Model file for the job. Use its own axes, mm. Coordinates: 2 decimals unless noted, no trailing zeros. Order: outer loops, then holes, each group sorted by start corner. A loop starts at its lowest first (then second) coordinate and runs counter-clockwise, first axis right, second up.
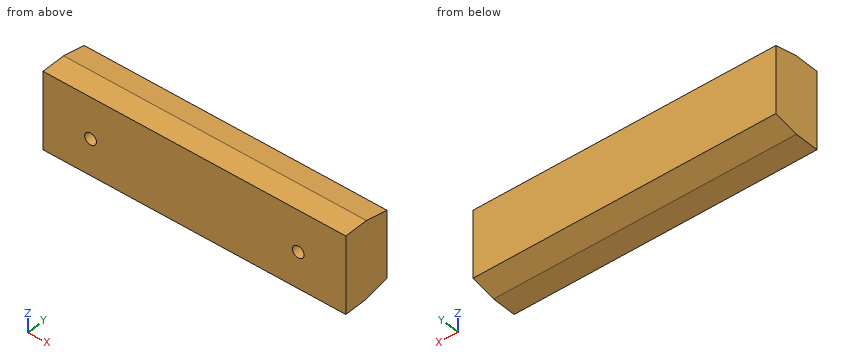
from build123d import *

# Parameters (mm, degrees)
SKETCH1_W             = 175
SKETCH1_H             = 28
BOSS_EXTRUDE1_DEPTH   = 45
M8_TAPPED_HOLE1_D     = 6.8
M8_TAPPED_HOLE1_DEPTH = 19.75
M8_TAPPED_HOLE1_TIP   = 2.042926105
CUT_EXTRUDE1_DEPTH    = 183.849665026


with BuildPart() as part:
    # Sketch1 → Boss-Extrude1 (new body)
    with BuildSketch(Plane.XY):
        with Locations((87.5, -14)):
            Rectangle(SKETCH1_W, SKETCH1_H)
    extrude(amount=BOSS_EXTRUDE1_DEPTH)

    # M8 Tapped Hole1
    with Locations(Plane(origin=(0, -28, 0), x_dir=(-1, 0, 0), z_dir=(0, -1, 0))):
        with Locations((-27.5, -21), (-147.5, -21)):
            Hole(M8_TAPPED_HOLE1_D / 2, depth=M8_TAPPED_HOLE1_DEPTH)
            with Locations((0, 0, -(M8_TAPPED_HOLE1_DEPTH + M8_TAPPED_HOLE1_TIP / 2))):  # 118° drill point
                Cone(0, M8_TAPPED_HOLE1_D / 2, M8_TAPPED_HOLE1_TIP, mode=Mode.SUBTRACT)

    # Sketch7 → Cut-Extrude1 (cut, through all)
    with BuildSketch(Plane.ZY):
        Polygon((3, 0), (0, -14), (0, 0), align=None)
        Polygon((45, 0), (42, 0), (45, -14), align=None)
    extrude(amount=-CUT_EXTRUDE1_DEPTH, mode=Mode.SUBTRACT)


solid = part.part
Q1. Probe line 1 (X direction, y = -20.25, z = 21); line 2 (Z direction, x = 147.5, y = -15.5); line 3 (X direction, y = -16.75, z = 22.5). List the from-to ranges inside material, lowest first.
Established:
line 1: x = 0 to 24.1, 30.9 to 144.1, 150.9 to 175
line 2: z = 0 to 17.6, 24.4 to 45
line 3: x = 0 to 24.45, 30.55 to 144.45, 150.55 to 175
Q2. Drop flat-ended pins along their axis: P1, Ø6, axis at x = 147.5, z = 21, coming from the -Y side; P2, Ø1.5, axis at x = 55, y = -3, coming from the +Z side; P3, Ø12, axis at x = 81.5, y = -5, coming from the +Z side. Give the stop position or say it passes through.
Established:
P1: stops at y = -8.01
P2: stops at z = 42.8
P3: stops at z = 44.36
Q3. Cut at B-B, the plane y = -4.5. List the corners of the cut face in (x, z).
Established:
outline: (0, 2.04) - (175, 2.04) - (175, 42.96) - (0, 42.96) - close
Q4. Cut at A-A, the plane x = 134.5. List the corners of the cut face in (y, z).
Established:
outline: (-28, 0) - (-14, 0) - (0, 3) - (0, 42) - (-14, 45) - (-28, 45) - close
